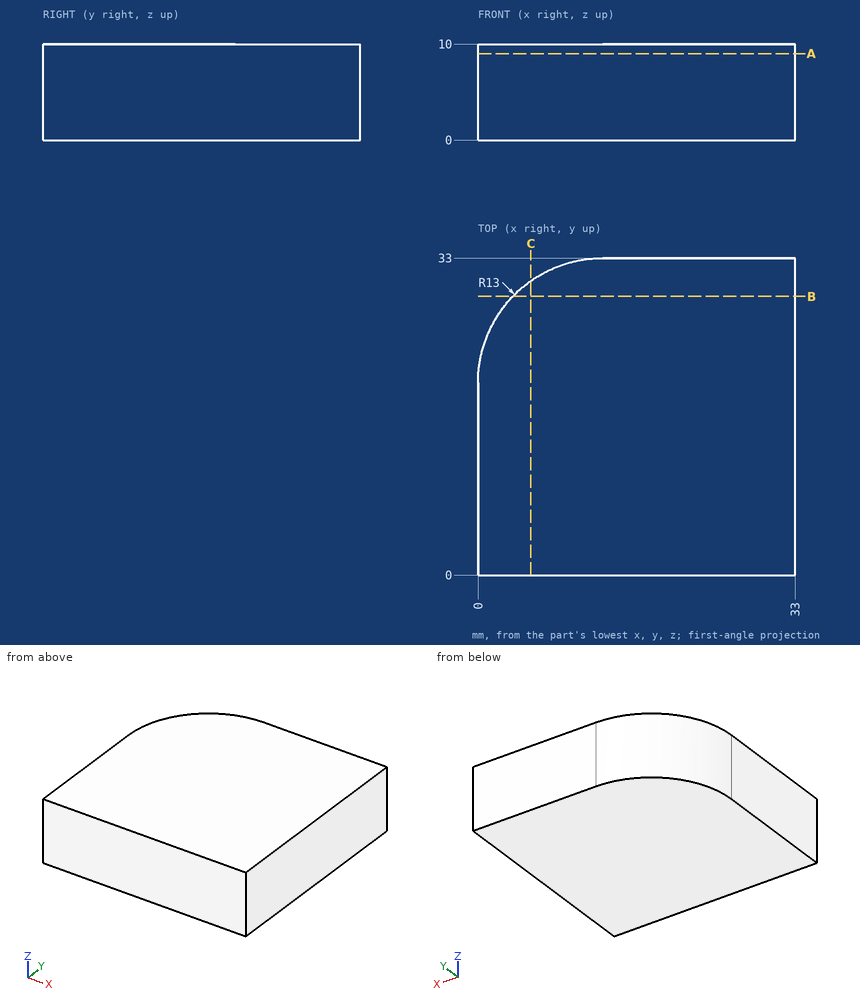
Input: dimensioned drawing with shaded views. Units: mm. Origin: part minimum x, y, z. Give positions to 0.01 mm unless a question says otherwise; leave off trailing zeros. Loops run counter-clockwise (first coordinate to the right, second up) from the corner with the lowest first, then second, coordinate; pieces in that order, holes last. Notation, with made-up numbers: M -30,57 L 5,57 A28 cw 5,84 Z; hole C -7.5,5 d1. An arc over 180 degrees is marked long. Put each result on its own line as item: value. Start each with the question number.
1) Cut plane A-A (z = 9). Output: boundary loops of the cut face in (x, y), then the cut area to 3 significant figures.
2) Cut plane B-B (y = 29). Output: boundary loops of the cut face in (x, z), then the cut area to 3 significant figures.
3) Contact query for a flat-ended pin moving along its axis: pin 1 (1 mm diameter, centred on y = 21, z = 2, fed in from -X). Output: stop coordinate, or through.
4) Ray query, line 1 along X through (y, z) = (24.5, 0.5); line 2 along X through (y, z) = (29, 8.75); line 3 along Y through (x, z) = (11, 3). Return the intervals inside material, ascending.
5) Cut plane C-C (x = 5.5). Output: boundary loops of the cut face in (y, z), then the cut area to 3 significant figures.
Verdict:
1. outline: M 0,0 L 33,0 L 33,33 L 13,33 A13 ccw 0,20 Z
1. area: 1,050 mm2
2. outline: M 3.62,0 L 33,0 L 33,10 L 3.62,10 Z
2. area: 294 mm2
3. pin 1: x = 0.01
4. line 1: 0.8 to 33
4. line 2: 3.62 to 33
4. line 3: 0 to 32.85
5. outline: M 0,0 L 30.62,0 L 30.62,10 L 0,10 Z
5. area: 306 mm2
